Answer from the drawing. Dimensions are ordinates in mm from the lowest x, y and z of the part. A direction names the side the tool comes from. Coordinates: 2 decimals unless noted, no trailing zeros. Order: outer loops, then holes, each group sorted by start corner. A loop starts at its lowest first (then second) coordinate and runs counter-clockwise, first axis right, second up. Notation, with made-up numbers: M 14.25,47 L 61.25,47 A16 cw 61.25,70 Z; hole C 68,25 d9. An arc over 180 degrees is marked long. Write each question's results on one line, items separated by ' | '.
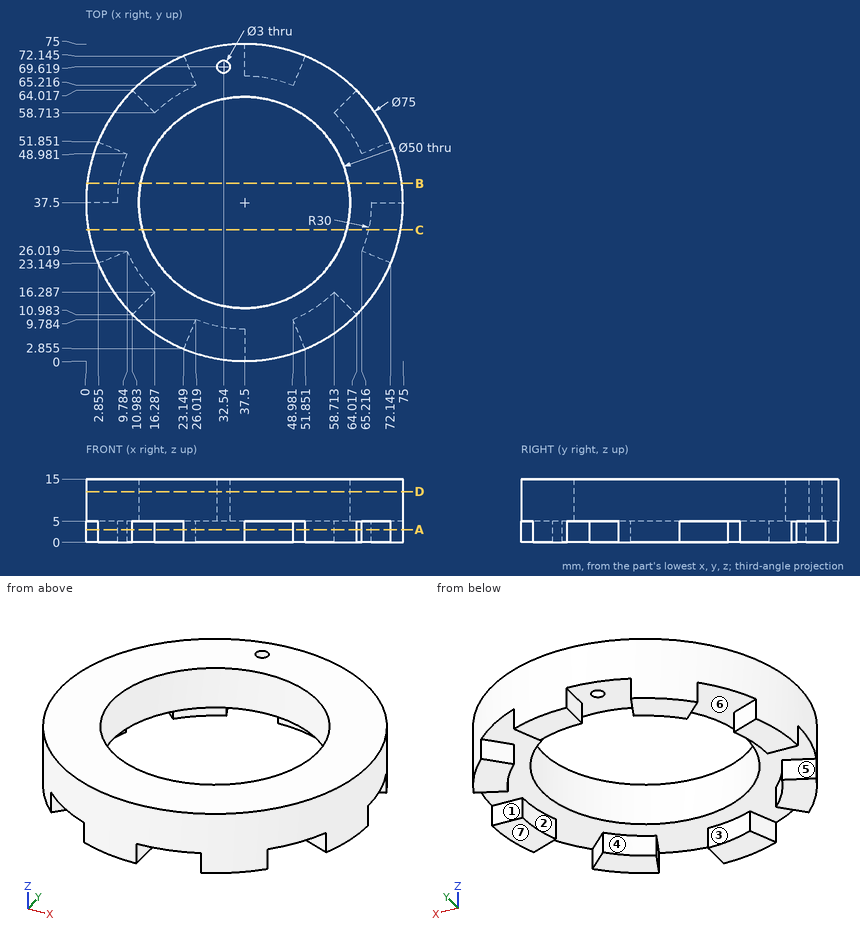
(1) Given pin 1 (6 mm diameter, centred on x = 59.5, z = 5.5, fed in from +Y); pin 2 (1.5 mm diameter, centred on y = 72.5, z = 3.5, fed in from -X); pin 3 (2 mm diameter, centred on x = 45, z = 7.5, fed in from +Y), each flat-ended and moving along its own axis, determine where each tip first touches the part or whether it passes through.
Conclusion:
pin 1: y = 69.83 | pin 2: x = 22.23 | pin 3: y = 74.43
(2) For the marked faces 1, 2, 3 and 4, determine the directions among +Z, -Z, +X, -X, +Y, -Y from which every point of the face is accessible in a straight line to the end or side of a thin tool.
Conclusion:
face 1: -Z, +X | face 2: -Z, -X | face 3: -Z, +Y | face 4: -Z
(3) The part is cut by section D-D, the plane z = 12. Write down the section's boundary in (x, y).
Conclusion:
outline: C 37.5,37.5 d75; hole C 37.5,37.5 d50; hole C 32.54,69.62 d3
(4) The mould has two halves that part along X. Classify the marked faces 5, 6 and 7: pulls with the +X half, pulls with the -X half, needs draft (parallel to the pull), parting line crosses it, or undercut.
Conclusion:
face 5: pulls with the -X half | face 6: undercut | face 7: needs draft
(5) The part is cut by section A-A, the plane z = 3. Count the separate pieces of the cut face and the enclosed holes in it.
Conclusion:
separate pieces: 8 | enclosed holes: 0
(6) The part is cut by section B-B, the plane y = 42. Write down the section's boundary in (x, z).
Conclusion:
outline: M 0.27,0 L 7.84,0 L 7.84,5 L 12.91,5 L 12.91,15 L 0.27,15 Z; M 62.09,5 L 74.73,5 L 74.73,15 L 62.09,15 Z
(7) The part is cut by section C-C, the plane y = 31. Write down the section's boundary in (x, z), then the cut area to 3 significant figures.
Conclusion:
outline: M 0.57,5 L 13.36,5 L 13.36,15 L 0.57,15 Z; M 61.64,5 L 66.79,5 L 66.79,0 L 74.43,0 L 74.43,15 L 61.64,15 Z | area: 294 mm²
(8) Straight lines are drawn through the part: line 1 (Y direction, x = 37.5, z = 11.25); line 2 (Y direction, x = 32.5, z = 10.5) (1 decimal); line 3 (Y direction, x = 23, z = 8) (1 decimal). For each, find the intervals that lie inside material, in ascending order.
Conclusion:
line 1: 0 to 12.5, 62.5 to 75 | line 2: 0.3 to 13, 62 to 68.1, 71.1 to 74.7 | line 3: 2.9 to 17.1, 57.9 to 72.1
